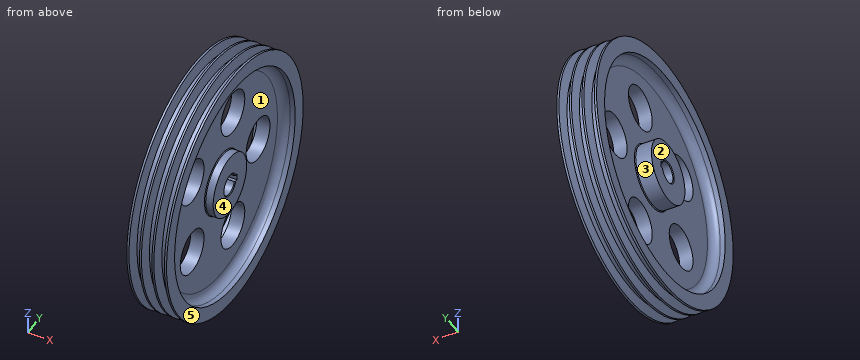
from build123d import *

# Parameters (mm, degrees)
SKETCH8_R           = 37.5
SKETCH8_R_2         = 12.5
BOSS_EXTRUDE2_DEPTH = 4
CUT_EXTRUDE5_REACH  = 224.535
SKETCH9_W           = 8
SKETCH9_H           = 6.6
CUT_EXTRUDE6_START  = -16
SKETCH10_R          = 135
SKETCH10_R_2        = 37.5
CUT_EXTRUDE6_DEPTH  = 16
SKETCH11_R          = 135
SKETCH11_R_2        = 37.5
CUT_EXTRUDE7_DEPTH  = 16
FILLET1_R           = 10
CHAMFER1_SIZE       = 1
SKETCH13_R          = 37.5
CUT_EXTRUDE9_DEPTH  = 6
CHAMFER2_SIZE       = 1
CUT_EXTRUDE8_REACH  = 220.728
SKETCH12_R          = 26.65
CIRPATTERN1_COUNT   = 5


with BuildPart() as part:
    # Sketch1 → Revolve1 (revolve)
    with BuildSketch(Plane.XY, mode=Mode.PRIVATE) as revolve1_sk:
        Polygon((6.128194326, 141.5), (2.61229149, 153), (0, 153), (0, 12.5), (48, 12.5), (48, 153), (45.38770851, 153), (41.871805674, 141.5), (36.191805674, 141.5), (32.675902837, 153), (30.355902837, 153), (26.84, 141.5), (21.16, 141.5), (17.644097163, 153), (15.324097163, 153), (11.808194326, 141.5), align=None)
    revolve(revolve1_sk.sketch.rotate(Axis((0, 0, 0), (1, 0, 0)), 270), axis=Axis((0, 0, 0), (1, 0, 0)))

    # Sketch8 → Boss-Extrude2 (add)
    with BuildSketch(Plane.ZY):
        Circle(SKETCH8_R)
        with Locations(Location((0, 0, 0), (0, 0, 180))):
            Circle(SKETCH8_R_2, mode=Mode.SUBTRACT)
    extrude(amount=BOSS_EXTRUDE2_DEPTH)

    # Sketch9 → Cut-Extrude5 (cut, up to next)
    with BuildSketch(Plane.ZY.offset(4), mode=Mode.PRIVATE) as cut_extrude5_sk1:
        with Locations((0, 12.5)):
            Rectangle(SKETCH9_W, SKETCH9_H)
    cut_extrude5_tool1 = extrude(cut_extrude5_sk1.sketch, amount=-CUT_EXTRUDE5_REACH, mode=Mode.PRIVATE) & part.part
    add(cut_extrude5_tool1.solids().sort_by_distance((-4, 12.5, 0))[0], mode=Mode.SUBTRACT)

    # Sketch10 → Cut-Extrude6 (cut)
    with BuildSketch(Plane.ZY.offset(CUT_EXTRUDE6_START)):
        Circle(SKETCH10_R)
        Circle(SKETCH10_R_2, mode=Mode.SUBTRACT)
    extrude(amount=CUT_EXTRUDE6_DEPTH, mode=Mode.SUBTRACT)

    # Sketch11 → Cut-Extrude7 (cut)
    with BuildSketch(Plane(origin=(48, 0, 0), x_dir=(0, 0, -1), z_dir=(1, 0, 0))):
        with Locations(Location((0, 0, 0), (0, 0, 180))):
            Circle(SKETCH11_R)
        with Locations(Location((0, 0, 0), (0, 0, 180))):
            Circle(SKETCH11_R_2, mode=Mode.SUBTRACT)
    extrude(amount=-CUT_EXTRUDE7_DEPTH, mode=Mode.SUBTRACT)

    # Fillet1
    fillet1_edges = [part.edges().sort_by_distance(p)[0] for p in [
        (16, 0, -135),
        (32, 0, -135),
    ]]
    fillet(fillet1_edges, radius=FILLET1_R)

    # Chamfer1
    chamfer1_edges = [part.edges().sort_by_distance(p)[0] for p in [
        (16, 0, -37.5),
        (32, 0, -37.5),
    ]]
    chamfer(chamfer1_edges, length=CHAMFER1_SIZE)

    # Sketch13 → Cut-Extrude9 (cut)
    with BuildSketch(Plane(origin=(48, 0, 0), x_dir=(0, 0, -1), z_dir=(1, 0, 0))):
        Circle(SKETCH13_R)
    extrude(amount=-CUT_EXTRUDE9_DEPTH, mode=Mode.SUBTRACT)

    # Chamfer2
    chamfer2_edges = [part.edges().sort_by_distance(p)[0] for p in [
        (-4, -12.5, 0),
        (42, -12.5, 0),
    ]]
    chamfer(chamfer2_edges, length=CHAMFER2_SIZE)

    # Sketch12 → Cut-Extrude8 (cut, up to next)
    with BuildSketch(Plane.ZY.offset(-16), mode=Mode.PRIVATE) as cut_extrude8_sk1:
        with Locations((0, 81.65)):
            Circle(SKETCH12_R)
    cut_extrude8_tool1 = extrude(cut_extrude8_sk1.sketch, amount=-CUT_EXTRUDE8_REACH, mode=Mode.PRIVATE) & part.part
    cut_extrude8 = cut_extrude8_tool1.solids().sort_by_distance((16, 81.65, 0))[0]
    add(cut_extrude8, mode=Mode.SUBTRACT)

    # CirPattern1: Cut-Extrude8 ×5 about axis
    cirpattern1_axis = Axis((0, 0, 0), (1, 0, 0))
    for i in range(1, CIRPATTERN1_COUNT):
        add(cut_extrude8.rotate(cirpattern1_axis, i * 360 / CIRPATTERN1_COUNT), mode=Mode.SUBTRACT)


solid = part.part
The listing builds one solid part. Answer for the finished solid, in the listing's coordinates (mm). Face numbers are marked on the shaded views. A direction names the side the tool comes from. Round coordinates to 2 decimals unless told otherwise and drop trailing zeros. Answer in a Markdown table with one row per item. Add a question column.
1) Which of the six approach directions +Z, -Z, +X, -X, +Y, -Y give full straight-line access (tool end or side, diameter ignored) to the marked faces 3, 4 and 5?
2) Flat-ended cylindrical pins translate along their axes: pin 1 Ø22.5 at (y, z) = (-10.5, 3) entering from +X; pin 2 Ø1.2 at (x, y) = (16, 14) entering from +Z; pin 3 Ø12 at (x, y) = (38.5, 18.5) entering from -Z. Find the tip coordinate at first contact, or state that the pin passes through.
3) The part is cut by section A-A on z = 0. Count the separate pieces of the cut face and the enclosed holes in it, plus the area to 3 significant figures.
4) Consider line 1 along Z through (x, y) = (1, -10); line 2 along X through (y, z) = (-111, 96.5); line 3 along X through (y, z) = (-110, 45). Determine where each line is inside the solid, lowest interval first. Write a range as from..to.
5) Determine the mould class of the marked faces 1 and 2 for opening direction Y: pulls with the +Y half, pulls with the -Y half, needs draft (parallel to the pull), parting line crosses it, or undercut.
Findings below:
| question | item | result |
|---|---|---|
| 1 | face 3 | -X |
| 1 | face 4 | +X |
| 1 | face 5 | +Z, -Z, +X, +Y, -Y |
| 2 | pin 1 | stops at x = 42 |
| 2 | pin 2 | stops at z = 152.41 |
| 2 | pin 3 | stops at z = -152.05 |
| 3 | separate pieces | 3 |
| 3 | enclosed holes | 0 |
| 3 | area | 5,600 mm² |
| 4 | line 1 | z = -152.67..-134.63, -36.14..-7.5, 7.5..36.14, 134.63..152.67 |
| 4 | line 2 | x = 0..4.42, 13.51..19.45, 28.55..34.49, 43.58..48 |
| 4 | line 3 | x = 16..32 |
| 5 | face 1 | undercut |
| 5 | face 2 | needs draft |
